Check sheet for the modelled part. Datum: model origin and axes. Units: mm. Face numbers are marked on the shaded views. A direction names the side the tool comes from. Give positions to 0.01 mm unless a question says otherwise; leave off trailing zeros. Loops run counter-clockwise (first coordinate to the right, second up) from the corner with the lowest first, then second, coordinate; pieces in that order, holes last. Notation, with made-up numbers: (45, 47.5) - (87, 47.5) arc R35 ccw to (87, 83.5) - close; hole circle Ø9 at (-30.75, -6). An arc over 180 degrees is marked (long way). Answer in a Markdown table with one row per item. Add a question column.
(1) Go/stop test with flat-tipped pins: P1, Ø3, axis at x = -1, y = 113.5, coming from the +Z side; P2, Ø4, axis at x = 1, y = 73.5, coming from the +Z side; P3, Ø6, axis at x = 4, y = 79, coming from the +Z side; P4, Ø1.5, axis at y = 86.5, z = -2.5, coming from the +X side. Record where each tip stops, or that it passes through.
(2) Thickness scan on L1, parallel to X at y = 92, z = 0; L2, parallel to Y at x = -4, z = 3.5; L3, parallel to Y at x = 3.75, z = -3.25. Record the ranges inside material, lowest first.
(3) Draft check along X on the marked faces 1, 2 and 3. Enter one of: released by +X, released by -X, zero draft, split by the parting line, or undercut.
(4) Sectioned sample at A-A on y = 113. Enter the section's corners in (x, z), then the cut area to 3 significant figures.
(5) Set-up check for the marked faces 4, 5 and 6: record each of +Z, -Z, +X, -X, +Y, -Y from which the full face is reachable in a straight line by a thin tool's end or side.
from build123d import *

# Parameters (mm, degrees)
BOSS_EXTRUDE1_DEPTH = 10.7
SKETCH3_W           = 4
SKETCH3_H           = 4.3


with BuildPart() as part:
    # Sketch1 → Revolve1 (revolve)
    with BuildSketch(Plane.XY, mode=Mode.PRIVATE) as revolve1_sk:
        Polygon((0, 110), (6.3865, 110), (7, 109.3865), (7, 60.6135), (6.3865, 60), (4, 60), (4, 50), (0, 50), align=None)
    revolve(revolve1_sk.sketch.rotate(Axis((0, 50, 0), (0, 1, 0)), 270), axis=Axis((0, 50, 0), (0, 1, 0)))

    # Sketch2 → Boss-Extrude1 (add)
    with BuildSketch(Plane(origin=(0, 110, 0), x_dir=(1, 0, 0), z_dir=(0, 1, 0))):
        Polygon((-5.773502692, 0), (-2.886751346, -5), (2.886751346, -5), (5.773502692, 0), (2.886751346, 5), (-2.886751346, 5), align=None)
    extrude(amount=BOSS_EXTRUDE1_DEPTH)

    # Sketch3 → Revolve2 (revolve)
    with BuildSketch(Plane.XY, mode=Mode.PRIVATE) as revolve2_sk:
        with Locations((2, 122.85)):
            Rectangle(SKETCH3_W, SKETCH3_H)
    revolve(revolve2_sk.sketch.rotate(Axis((0, 120.7, 0), (0, 1, 0)), 270), axis=Axis((0, 120.7, 0), (0, 1, 0)))

    # Sketch4 → Cut-Revolve1 (revolve, cut)
    with BuildSketch(Plane.XY, mode=Mode.PRIVATE) as cut_revolve1_sk:
        Polygon((0, 125), (2.5, 125), (2.067, 124.567), (2.067, 120), (2, 119.961317532), (2, 50), (0, 50), align=None)
    revolve(cut_revolve1_sk.sketch.rotate(Axis((0, 50, 0), (0, 1, 0)), 270), axis=Axis((0, 50, 0), (0, 1, 0)), mode=Mode.SUBTRACT)


solid = part.part
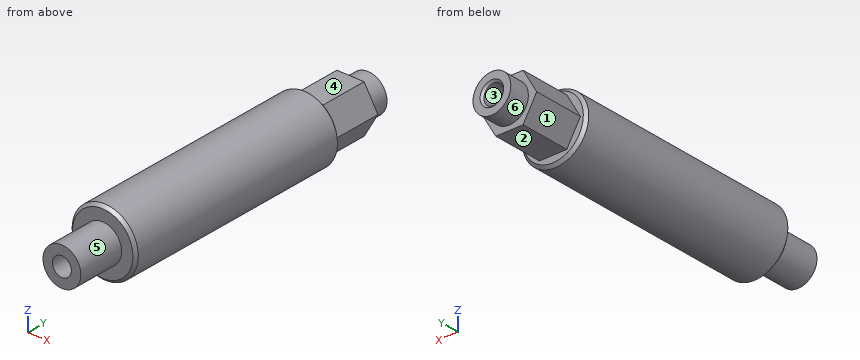
Reply:
| question | item | result |
|---|---|---|
| 1 | P1 | z = 5 |
| 1 | P2 | z = 7 |
| 1 | P3 | z = 6.93 |
| 1 | P4 | x = 6.78 |
| 2 | L1 | -7 to -2, 2 to 7 |
| 2 | L2 | 60 to 110 |
| 2 | L3 | 60 to 120.7 |
| 3 | face 1 | released by -X |
| 3 | face 2 | zero draft |
| 3 | face 3 | undercut |
| 4 | outline | (-5.77, 0) - (-2.89, -5) - (2.89, -5) - (5.77, 0) - (2.89, 5) - (-2.89, 5) - close; hole circle Ø4 at (0, 0) |
| 4 | area | 74.0 mm^2 |
| 5 | face 4 | +Z, +X, -X, +Y |
| 5 | face 5 | -Y |
| 5 | face 6 | +Y |
